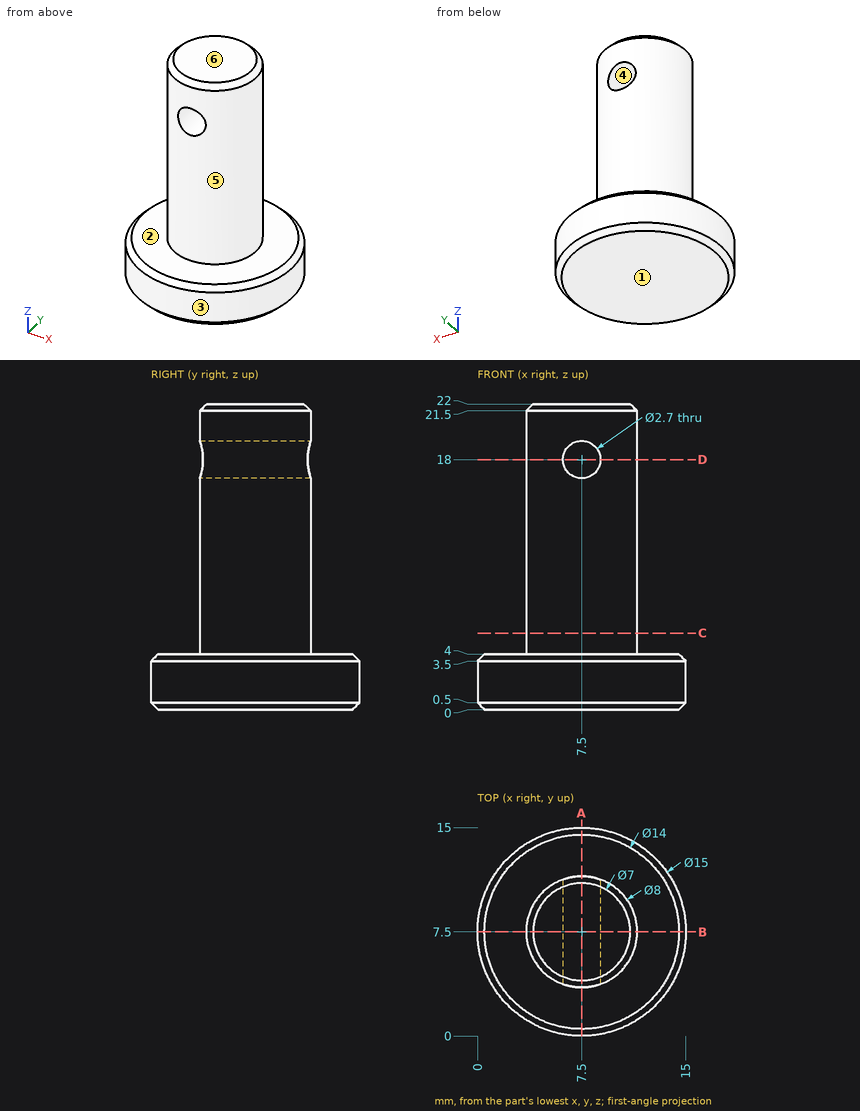
Source: three-view drawing plus pictorial views. Frame: mm from the lowest corner of the part. A direction names the side the tool comes from. Round coordinates to 2 decimals unless told otherwise and drop trailing zeros. Loops run counter-clockwise (first coordinate to the right, second up) from the corner with the lowest first, then second, coordinate; pieces in that order, holes last. Notation, with made-up numbers: (23, 64) - (66, 64) arc R20 cw to (66, 87) - close; hole circle Ø9 at (38.25, 67.5). An arc over 180 degrees is marked (long way). Write each question's results on one line, items separated by ' | '. Start each with the question number.
1) Cut plane C-C on z = 5.5. Return loops of the section in (x, y).
2) Cut plane B-B on y = 7.5. Return loops of the section in (x, z).
3) Cut plane A-A on x = 7.5. Return loops of the section in (y, z), then the cut area to 3 significant figures.
4) Mould query, pull axis Z, two halves, no side actions, for the marked faces 1, 2, 3 and 4. Classes: released by +Z, released by -Z, zero draft, split by the parting line, or undercut.
5) Access query for the marked faces 5 and 6. Directions: +Z, -Z, +X, -X, +Y, -Y. A direction counts if a zero-diameter tool reaches every point of the face in a straight line with its end or side. Return the directions, or none.
6) Cut plane D-D on z = 18. Return loops of the section in (x, y).
7) First-contact query: P1, Ø5, axis at x = 2.5, y = 5, coming from the +Z side; P2, Ø5, axis at y = 11, z = 3.5, coming from the +X side; P3, Ø1.5, axis at x = 6.5, z = 6, coming from the +Y side; P4, Ø4, axis at x = 4, z = 12.5, coming from the +Y side. Flat tips, straight axial feed; report the tip coordinate or a pass-through.
8) Line query: probe 1 along Z at (x, y) = (7.5, 8); probe 2 along X at (y, z) = (9, 18); probe 3 along Z at (x, y) = (8, 2.5). Output: solid intervals per line, ascending. Write a range as [from, to].
Verdict:
1) outline: circle Ø8 at (7.5, 7.5)
2) outline: (0, 0.5) - (0.5, 0) - (14.5, 0) - (15, 0.5) - (15, 3.5) - (14.5, 4) - (11.5, 4) - (11.5, 21.5) - (11, 22) - (4, 22) - (3.5, 21.5) - (3.5, 4) - (0.5, 4) - (0, 3.5) - close; hole circle Ø2.7 at (7.5, 18)
3) outline: (0, 0.5) - (0.5, 0) - (14.5, 0) - (15, 0.5) - (15, 3.5) - (14.5, 4) - (11.5, 4) - (11.5, 16.65) - (3.5, 16.65) - (3.5, 4) - (0.5, 4) - (0, 3.5) - close; (3.5, 19.35) - (11.5, 19.35) - (11.5, 21.5) - (11, 22) - (4, 22) - (3.5, 21.5) - close | area: 182 mm2
4) face 1: released by -Z | face 2: released by +Z | face 3: zero draft | face 4: undercut
5) face 5: +Z | face 6: +Z, +X, -X, +Y, -Y
6) outline: (6.15, 3.73) - (6.15, 11.27) arc R4 ccw to start; (8.85, 3.73) arc R4 ccw to (8.85, 11.27) - close
7) P1: stops at z = 22 | P2: stops at x = 14.93 | P3: stops at y = 11.49 | P4: stops at y = 11.21
8) probe 1: z = [0, 16.65], [19.35, 22] | probe 2: x = [3.79, 6.15], [8.85, 11.21] | probe 3: z = [0, 4]
